For this review, take the finished solid that the model builds, in its own axes (mm). Face numbers are marked on the shaded views. Give positions to 0.01 mm unless a question says otherwise; leave off trailing zeros. Order: outer loops, then holes, each group sorted by start corner. A loop starts at its lowest first (then second) coordinate and runs counter-clockwise, first axis right, second up.
Item 1: The part is to be moulded in two halves that separate along Y. For the marked faces 1, 2 and 3, say which applies: released by +Y, released by -Y, zero draft, split by the parting line, or undercut.
Item 2: Consider section B-B (z = 4.75). Give the boundary of the cut face in (x, y), plus the area to 3 significant figures.
Item 3: For P1, Ø7, axis at x = 16, y = 16, coming from the +Z side; P2, Ø7, axis at x = 110, y = 110, coming from the -Z side, all flat-tipped, find the tip position at first contact; note any pin that passes through.
Item 4: For probe 1 along Y at (x, z) = (16, 7.5); probe 2 along Y at (x, z) = (110.5, 11), list the stretches that pass through material, from the lowest coordinate up.
Item 5: Consider section A-A (y = 63). Give the boundary of the cut face in (x, z).
```python
from build123d import *

# Parameters (mm, degrees)
SKETCH1_R                  = 55
BOSS_EXTRUDE1_DEPTH        = 20
SKETCH2_R                  = 60
SKETCH2_R_2                = 55
BOSS_EXTRUDE2_DEPTH        = 2.5
M10X1_5_TAPPED_HOLE1_D     = 8.5
M10X1_5_TAPPED_HOLE1_DEPTH = 12
M10X1_5_TAPPED_HOLE1_TIP   = 2.553657631
CHAMFER1_SIZE              = 1


with BuildPart() as part:
    # Sketch1 → Boss-Extrude1 (new body)
    with BuildSketch(Plane.XY):
        with BuildLine():
            Line((16, 0), (110, 0))
            ThreePointArc((110, 0), (121.313708499, 4.686291501), (126, 16))
            Line((126, 16), (126, 110))
            ThreePointArc((126, 110), (121.313708499, 121.313708499), (110, 126))
            Line((110, 126), (16, 126))
            ThreePointArc((16, 126), (4.686291501, 121.313708499), (0, 110))
            Line((0, 110), (0, 16))
            ThreePointArc((0, 16), (4.686291501, 4.686291501), (16, 0))
        make_face()
        with Locations((63, 63)):
            Circle(SKETCH1_R, mode=Mode.SUBTRACT)
    extrude(amount=BOSS_EXTRUDE1_DEPTH)

    # Sketch2 → Boss-Extrude2 (add)
    with BuildSketch(Plane.XY.offset(20)):
        with Locations((63, 63)):
            Circle(SKETCH2_R)
        with Locations((63, 63)):
            Circle(SKETCH2_R_2, mode=Mode.SUBTRACT)
    extrude(amount=BOSS_EXTRUDE2_DEPTH)

    # M10x1.5 Tapped Hole1
    with Locations(Plane(origin=(110, 110, 0), x_dir=(-1, 0, 0), z_dir=(0, 0, -1))):
        with Locations((0, 0), (94, 0), (94, -94), (0, -94)):
            Hole(M10X1_5_TAPPED_HOLE1_D / 2, depth=M10X1_5_TAPPED_HOLE1_DEPTH)
            with Locations((0, 0, -(M10X1_5_TAPPED_HOLE1_DEPTH + M10X1_5_TAPPED_HOLE1_TIP / 2))):  # 118° drill point
                Cone(0, M10X1_5_TAPPED_HOLE1_D / 2, M10X1_5_TAPPED_HOLE1_TIP, mode=Mode.SUBTRACT)

    # Chamfer1
    chamfer1_edges = [part.edges().sort_by_distance(p)[0] for p in [
        (8, 63, 0),
    ]]
    chamfer(chamfer1_edges, length=CHAMFER1_SIZE)


solid = part.part
```
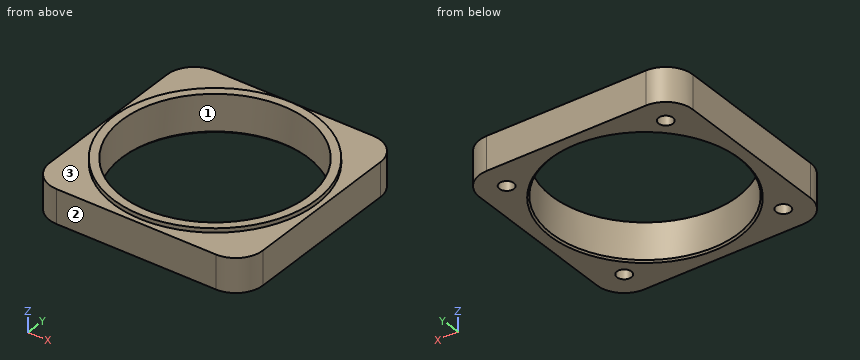
Resolved:
1. face 1: undercut
1. face 2: released by -Y
1. face 3: zero draft
2. outline: (0, 16) arc R16 ccw to (16, 0) - (110, 0) arc R16 ccw to (126, 16) - (126, 110) arc R16 ccw to (110, 126) - (16, 126) arc R16 ccw to (0, 110) - close; hole circle Ø110 at (63, 63); hole circle Ø8.5 at (16, 16); hole circle Ø8.5 at (16, 110); hole circle Ø8.5 at (110, 16); hole circle Ø8.5 at (110, 110)
2. area: 5,930 mm2
3. P1: stops at z = 20
3. P2: stops at z = 12.45
4. probe 1: y = 0 to 11.75, 20.25 to 34.43, 91.57 to 105.75, 114.25 to 126
4. probe 2: y = 0.01 to 11.78, 20.22 to 35.27, 90.73 to 105.78, 114.22 to 125.99
5. outline: (0, 0) - (7, 0) - (8, 1) - (8, 22.5) - (3, 22.5) - (3, 20) - (0, 20) - close; (118, 1) - (119, 0) - (126, 0) - (126, 20) - (123, 20) - (123, 22.5) - (118, 22.5) - close
